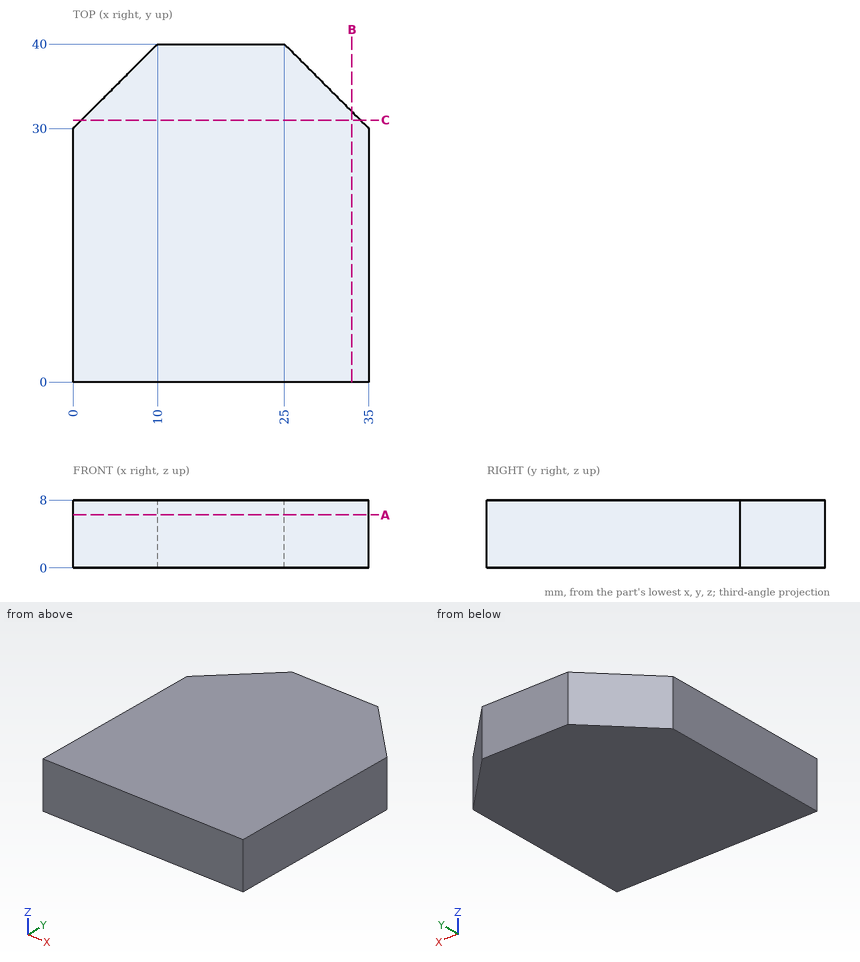
Drawing for the job (mm, zero at the part's lowest x, y, z). Round coordinates to 2 decimals unless told otherwise and drop trailing zeros. Write each loop counter-clockwise with the first axis right and the second up, starting at its lowest first coordinate (ties: lowest second). Pieces come first, ordered by that corner, then holes. Notation, with made-up numbers: (12.5, 34) - (61.5, 34) arc R30 ccw to (61.5, 65) - close; hole circle Ø6 at (63.5, 88). An arc over 180 degrees is marked (long way). Write item = value, one per line. Start each with the question number.
Q1. Band-saw the part on A-A (z = 6.25). Give the cut face in (x, y), then the cut area to 3 significant figures.
Q2. Band-saw the part on B-B (x = 33). Give the cut face in (y, z).
Q3. Band-saw the part on C-C (y = 31). Give the cut face in (x, z).
Q4. Probe L1, parallel to Y at x = 3.5, z = 3; L2, parallel to Y at x = 28, z = 2.5; L3, parallel to X at y = 38, z = 4.5. List the from-to ranges inside material, lowest first. Write a range as from..to.
Answers below:
q1.outline = (0, 0) - (35, 0) - (35, 30) - (25, 40) - (10, 40) - (0, 30) - close
q1.area = 1,300 mm2
q2.outline = (0, 0) - (32, 0) - (32, 8) - (0, 8) - close
q3.outline = (1, 0) - (34, 0) - (34, 8) - (1, 8) - close
q4.L1 = 0..33.5
q4.L2 = 0..37
q4.L3 = 8..27
